Read the model definition and answer for the solid it produces. Units are mm, in the model's axes. A direction names the side the tool comes from. Round coordinates to 2 decimals unless told otherwise and drop trailing zeros. Write each loop counter-clockwise with the first axis right and the second up, starting at its lowest first coordinate (ties: lowest second). Pieces come first, ordered by that corner, then holes. Notation, with made-up numbers: (-9.5, -6) - (12.5, -6) arc R25 cw to (12.5, 16) - close; hole circle Ø8 at (7.5, -28.75). An arc over 180 degrees is marked (long way). One line per item, written item: value. Start each with the question number.
(1) A cutting plane is placed at A-A, the plane x = 7. Determine the outline of the cut face in (y, z) (3 decimals).
(2) The mould has two halves that part along Z. Classify faces 1 (the face through (48.986, 4.056, -58.107)), 2 (the face through (58.107, 4.056, 48.986)), 3 (the face through (53.29, 5.01, -51.28)): +Z half, -Z half, draft (parallel to the pull), parting line (faces both ways), or undercut.
(3) Flat-ended cylindrical pins translate along their axes: pin 1 Ø1.5 at (y, z) = (1, -51) entering from +X; pin 2 Ø2 at (x, y) = (62, 2) entering from -Z; pin 3 Ø1.8 at (x, z) = (7, 50) entering from -Y; pin 4 Ø3 at (x, y) = (19, 4.5) entering from -Z. Find the tip coordinate at first contact, or state that the pin passes through.
(4) A cutting plane is placed at D-D, the plane z = 31.5. Determine the outline of the cut face in (x, y).
(5) For faces 4 (the face through (47.812, 4.056, 56.437)), 5 (the face through (20, 4, 0)), 6 (the face through (63.9, 4.1, 37.3)), determine the directions among +Z, -Z, +X, -X, +Y, -Y from which every point of the face is accessible in a straight line to the end or side of a thin tool.
(6) A cutting plane is placed at B-B, the plane x = 27. Determine the outline of the cut face in (y, z).
(7) Find the intervals of material crossed by L1, parallel to X at y = 5.25, z = -50; L2, parallel to X at y = 3.25, z = 50; L3, parallel to X at y = 6.25, z = -53.5, in increasing order.
(8) A cutting plane is placed at C-C, the plane z = -37.5. Determine the outline of the cut face in (x, y), plus the area to 3 significant figures.
from build123d import *

# Parameters (mm, degrees)
BOSS_EXTRUDE1_DEPTH = 8
SKETCH2_R           = 1.5
CUT_EXTRUDE1_DEPTH  = 101.727354775
BOSS_EXTRUDE2_START = -71
SKETCH3_W           = 8
SKETCH3_H           = 25
BOSS_EXTRUDE2_DEPTH = 5
SKETCH4_R           = 1.5
CUT_EXTRUDE2_DEPTH  = 5
CIRPATTERN1_COUNT   = 2
CIRPATTERN1_ANGLE   = 90
SKETCH5_R           = 1.55
CUT_EXTRUDE3_DEPTH  = 101.727354775


with BuildPart() as part:
    # Sketch1 → Boss-Extrude1 (new body)
    with BuildSketch(Plane(origin=(0, 0, 0), x_dir=(1, 0, 0), z_dir=(0, 1, 0))):
        with BuildLine():
            Line((0, -71), (0, -20))
            ThreePointArc((0, -20), (20, 0), (0, 20))
            Line((0, 20), (0, 71))
            ThreePointArc((0, 71), (71, 0), (0, -71))
        make_face()
    extrude(amount=BOSS_EXTRUDE1_DEPTH)

    # Sketch2 → Cut-Extrude1 (cut, through all)
    with BuildSketch(Plane(origin=(0, 8, 0), x_dir=(1, 0, 0), z_dir=(0, 1, 0))):
        with Locations(Location((7, 50, 0), (0, 0, 270))):
            Circle(SKETCH2_R)
        with Locations(Location((20, 50, 0), (0, 0, 270))):
            Circle(SKETCH2_R)
        with Locations(Location((20, -50, 0), (0, 0, 90))):
            Circle(SKETCH2_R)
        with Locations(Location((7, -50, 0), (0, 0, 90))):
            Circle(SKETCH2_R)
    extrude(amount=-CUT_EXTRUDE1_DEPTH, mode=Mode.SUBTRACT)

    # Sketch3 → Boss-Extrude2 (add, symmetric)
    with BuildSketch(Plane(origin=(0, 0, 0), x_dir=(0, -1, 0), z_dir=(-0.6427876096865403, 0, 0.7660444431189772)).offset(BOSS_EXTRUDE2_START)):
        with Locations((-4, 0)):
            Rectangle(SKETCH3_W, SKETCH3_H)
    boss_extrude2 = extrude(amount=BOSS_EXTRUDE2_DEPTH, both=True)

    # Sketch4 → Cut-Extrude2 (cut)
    with BuildSketch(Plane(origin=(48.851858336, 0, -58.219377677), x_dir=(-0.7660444431189771, 0, -0.6427876096865404), z_dir=(0.6427876096865404, 0, -0.7660444431189771))):
        with Locations((-6.75, 4)):
            Circle(SKETCH4_R)
        with Locations((6.75, 4)):
            Circle(SKETCH4_R)
    cut_extrude2 = extrude(amount=-CUT_EXTRUDE2_DEPTH, mode=Mode.SUBTRACT)

    # CirPattern1: Boss-Extrude2, Cut-Extrude2 ×2 about axis
    cirpattern1_axis = Axis((0, 0, 0), (0, -1, 0))
    add([boss_extrude2.rotate(cirpattern1_axis, i * CIRPATTERN1_ANGLE / (CIRPATTERN1_COUNT - 1)) for i in range(1, CIRPATTERN1_COUNT)])
    add([cut_extrude2.rotate(cirpattern1_axis, i * CIRPATTERN1_ANGLE / (CIRPATTERN1_COUNT - 1)) for i in range(1, CIRPATTERN1_COUNT)], mode=Mode.SUBTRACT)

    # Sketch5 → Cut-Extrude3 (cut, through all)
    with BuildSketch(Plane(origin=(0, 8, 0), x_dir=(1, 0, 0), z_dir=(0, 1, 0))):
        with Locations(Location((27, 0, 0), (0, 0, 270))):
            Circle(SKETCH5_R)
    extrude(amount=-CUT_EXTRUDE3_DEPTH, mode=Mode.SUBTRACT)


solid = part.part
Here are the results:
1. outline: (0, -70.654) - (8, -70.654) - (8, -51.5) - (0, -51.5) - close; (0, -48.5) - (8, -48.5) - (8, -18.735) - (0, -18.735) - close; (0, 18.735) - (8, 18.735) - (8, 48.5) - (0, 48.5) - close; (0, 51.5) - (8, 51.5) - (8, 70.654) - (0, 70.654) - close
2. face 1: -Z half
2. face 2: +Z half
2. face 3: undercut
3. pin 1: x = 58.35
3. pin 2: z = -36.33
3. pin 3: through
3. pin 4: z = -68.81
4. outline: (0, 0) - (63.63, 0) - (63.63, 8) - (0, 8) - close
5. face 4: +Z, +Y, -Y
5. face 5: -X, +Y, -Y
5. face 6: +X, +Y, -Y
6. outline: (0, -65.67) - (8, -65.67) - (8, -1.55) - (0, -1.55) - close; (0, 1.55) - (8, 1.55) - (8, 65.67) - (0, 65.67) - close
7. L1: 0 to 5.5, 8.5 to 18.5, 21.5 to 50.87, 51.85 to 58.27
7. L2: 0 to 5.5, 8.5 to 18.5, 21.5 to 50.73, 51.11 to 57.26
7. L3: 0 to 54.48
8. outline: (0, 0) - (60.29, 0) - (60.29, 8) - (0, 8) - close
8. area: 482 mm²
